The model under review builds one solid part; all positions refer to its coordinate system, in mm. A direction names the side the tool comes from. Coordinates: 2 decimals unless noted, no trailing zeros. Loops run counter-clockwise (first coordinate to the right, second up) from the corner with the lowest first, then second, coordinate; pieces in that order, holes last. Notation, with made-up numbers: (1, 70.5) - (32, 70.5) arc R16 ccw to (32, 89.5) - close; hole circle Ø1 at (-15, -31). An arc over 180 degrees is marked (long way). Answer in a Markdown table with one row per item. Add a question column.
(1) Machinability: for faces 1 (the conical face through (0.195, 4.649, -8.099)), 2 (the flat face through (7.5, 4, -6)), which of the approach directions +Z, -Z, +X, -X, +Y, -Y give a long, thin tool a straight path to every point of the face, cutting with its end or side? Answer none if there is none.
(2) For line 1 along X through (y, z) = (6.25, -6.25); line 2 along X through (y, z) = (6, 4.75); line 3 along Z through (x, y) = (41, 1.25), list the stretches that pass through material, from the lowest coordinate up.
(3) We need section A-A on x = 115. Write out the cut boundary in (y, z), plus the area to 3 significant figures.
(4) For P1, Ø2, axis at x = 25.5, z = 1.5, coming from the +Y side; P2, Ø4, axis at x = 16, y = 4, coming from the +Z side; P3, Ø6, axis at x = 73.5, y = 2, coming from the +Z side, all flat-tipped, find the tip position at first contact; note any pin that passes through.
from build123d import *

# Parameters (mm, degrees)
EXTRUDE_421_DEPTH = 7.5
FILLET_1347_R     = 0.6


with BuildPart() as part:
    # 草图1 → Extrude 421 (new body)
    with BuildSketch(Plane(origin=(0, 0, 0), x_dir=(0, 0, -1), z_dir=(1, 0, 0))):
        Polygon((9, 5.196152423), (9, -5.196152423), (0, -10.392304845), (-9, -5.196152423), (-9, 5.196152423), (0, 10.392304845), align=None)
    extrude(amount=EXTRUDE_421_DEPTH)

    # 草图2 → 凸台-旋转1 (revolve)
    with BuildSketch(Plane.XY, mode=Mode.PRIVATE) as revolve_1_sk:
        Polygon((0, 0), (127.5, 0), (127.5, 4.701), (127.5, 6), (63.75, 6), (0, 6), align=None)
    revolve(revolve_1_sk.sketch.rotate(Axis((0, 0, 0), (1, 0, 0)), 90), axis=Axis((0, 0, 0), (1, 0, 0)))

    # 草图3 → 切除-旋转1 (revolve, cut)
    with BuildSketch(Plane.XY):
        Polygon((0, 9), (3.690598923, 15.392304845), (3.690598923, 20.392304845), (-10, 20.392304845), (-10, 9), align=None)
    revolve(axis=Axis((0, 0, 0), (1, 0, 0)), mode=Mode.SUBTRACT)

    # 草图4 → 切除-旋转3 (revolve, cut)
    with BuildSketch(Plane.XY, mode=Mode.PRIVATE) as cut_revolve_3_sk:
        Polygon((7.5, 8.315), (6.9, 8.661410162), (6.9, 10.392304845), (7.5, 10.392304845), align=None)
    revolve(cut_revolve_3_sk.sketch.rotate(Axis((0, 0, 0), (1, 0, 0)), 90), axis=Axis((0, 0, 0), (1, 0, 0)), mode=Mode.SUBTRACT)

    # Fillet 1347
    fillet_1347_edges = [part.edges().sort_by_distance(p)[0] for p in [
        (7.5, 0, -6),
    ]]
    fillet(fillet_1347_edges, radius=FILLET_1347_R)

    # 草图6 → 切除-旋转4 (revolve, cut)
    with BuildSketch(Plane.XY, mode=Mode.PRIVATE) as cut_revolve_4_sk:
        Polygon((126.75, 6), (128.25, 6), (127.5, 4.700961894), align=None)
    revolve(cut_revolve_4_sk.sketch.rotate(Axis((0, 0, 0), (1, 0, 0)), 90), axis=Axis((0, 0, 0), (1, 0, 0)), mode=Mode.SUBTRACT)


solid = part.part
Outcome:
| question | item | result |
|---|---|---|
| 1 | face 1 | -Z, -X, +Y |
| 1 | face 2 | +X |
| 2 | line 1 | 0 to 6.9 |
| 2 | line 2 | 0 to 7.5 |
| 2 | line 3 | -5.87 to 5.87 |
| 3 | outline | circle Ø12 at (0, 0) |
| 3 | area | 113 mm² |
| 4 | P1 | y = 5.98 |
| 4 | P2 | z = 5.66 |
| 4 | P3 | z = 6 |
